Build history of the part. All positions in model axes, mm. Round coordinates to 2 decimals unless told otherwise and drop trailing zeros. Loops run counter-clockwise (first coordinate to the right, second up) from the corner with the lowest first, then second, coordinate; pieces in that order, holes last.
from build123d import *

# Parameters (mm, degrees)
SKETCH_1_W      = 60
SKETCH_1_H      = 35
SKETCH_1_R      = 3.3
EXTRUDE_1_DEPTH = 4
FILLET_1_R      = 3


with BuildPart() as part:
    # 草图1 → 凸台-拉伸1 (new body)
    with BuildSketch(Plane.XY):
        Rectangle(SKETCH_1_W, SKETCH_1_H)
        with Locations((-22.5, 0)):
            Circle(SKETCH_1_R, mode=Mode.SUBTRACT)
        with Locations((22.5, 0)):
            Circle(SKETCH_1_R, mode=Mode.SUBTRACT)
    extrude(amount=EXTRUDE_1_DEPTH)

    # 圆角1
    fillet_1_edges = [part.edges().sort_by_distance(p)[0] for p in [
        (30, -17.5, 2),
        (-30, -17.5, 2),
        (-30, 17.5, 2),
        (30, 17.5, 2),
    ]]
    fillet(fillet_1_edges, radius=FILLET_1_R)


solid = part.part
(1) Slice it at C-C on x = -22.5. List the corners of the cut face in (y, z), plus the area to 3 significant figures.
Responses:
outline: (-17.5, 0) - (-3.3, 0) - (-3.3, 4) - (-17.5, 4) - close; (3.3, 0) - (17.5, 0) - (17.5, 4) - (3.3, 4) - close
area: 114 mm2
(2) Probe line 1 (Y direction, x = -22.5, z = 0.9); line 2 (X direction, y = -1, z = 2.4); line 3 (X direction, y = 2, z = 3.85). List the from-to ranges inside material, lowest first.
Responses:
line 1: y = -17.5 to -3.3, 3.3 to 17.5
line 2: x = -30 to -25.64, -19.36 to 19.36, 25.64 to 30
line 3: x = -30 to -25.12, -19.88 to 19.88, 25.12 to 30
(3) Slice it at A-A on y = 0. List the corners of the cut face in (x, z).
Responses:
outline: (-30, 0) - (-25.8, 0) - (-25.8, 4) - (-30, 4) - close; (-19.2, 0) - (19.2, 0) - (19.2, 4) - (-19.2, 4) - close; (25.8, 0) - (30, 0) - (30, 4) - (25.8, 4) - close
(4) Pull direction X, two halves, no side cores. Call faces 1 (the face through (-29.14, 16.6, 2.03)), 2 (the face through (0, 0, 4)), 3 (the face through (29.1, -16.64, 2.03)), 4 (the face through (25.55, -1.26, 1.97)): +X half, -X half, draft (parallel to the pull), parting line (faces both ways), or undercut.
Responses:
face 1: -X half
face 2: draft
face 3: +X half
face 4: undercut
(5) Slice it at B-B on z = 2. List the corners of the cut face in (x, y).
Responses:
outline: (-30, -14.5) arc R3 ccw to (-27, -17.5) - (27, -17.5) arc R3 ccw to (30, -14.5) - (30, 14.5) arc R3 ccw to (27, 17.5) - (-27, 17.5) arc R3 ccw to (-30, 14.5) - close; hole circle Ø6.6 at (-22.5, 0); hole circle Ø6.6 at (22.5, 0)
(6) Slice it at D-D on x = 22. List the corners of the cut face in (y, z).
Responses:
outline: (-17.5, 0) - (-3.26, 0) - (-3.26, 4) - (-17.5, 4) - close; (3.26, 0) - (17.5, 0) - (17.5, 4) - (3.26, 4) - close
